```python
from build123d import *

# Parameters (mm, degrees)
BOSS_EXTRUDE1_DEPTH            = 5
SKETCH3_R                      = 4
BOSS_EXTRUDE2_DEPTH            = 5
CHAMFER1_SIZE                  = 1
M6X1_0_TAPPED_HOLE2_AT_2_COUNT = 2
M6X1_0_TAPPED_HOLE2_AT_2_PITCH = 0.000121298


with BuildPart() as part:
    # Sketch1 → Boss-Extrude1 (new, symmetric)
    with BuildSketch(Plane(origin=(0, 0, 0), x_dir=(1, 0, 0), z_dir=(0, 1, 0))):
        Polygon((0, 5.5), (-4.763139721, 2.75), (-4.763139721, -2.75), (0, -5.5), (4.763139721, -2.75), (4.763139721, 2.75), align=None)
    extrude(amount=BOSS_EXTRUDE1_DEPTH, both=True)

    # Sketch3 → Boss-Extrude2 (add)
    with BuildSketch(Plane(origin=(0, 5, 0), x_dir=(1, 0, 0), z_dir=(0, 1, 0))):
        with Locations(Location((0, 0, 0), (0, 0, 270))):
            Circle(SKETCH3_R)
    extrude(amount=BOSS_EXTRUDE2_DEPTH)

    # Chamfer1
    chamfer1_edges = [part.edges().sort_by_distance(p)[0] for p in [
        (0, 10, -4),
    ]]
    chamfer(chamfer1_edges, length=CHAMFER1_SIZE)

    # Sketch19 → M6x1.0 Tapped Hole2 (revolve, cut)
    with BuildSketch(Plane(origin=(-7.813e-06, -5, 0.000121047), x_dir=(0, 0, -1), z_dir=(1, 0, 0))):
        Polygon((0, 0), (0, 9.502151548), (2.5, 8), (2.5, 0), align=None)
    m6x1_0_tapped_hole2 = revolve(axis=Axis((-7.813e-06, -11.35, 0.000121047), (0, 1, 0)), mode=Mode.SUBTRACT)

    # M6x1.0 Tapped Hole2 at 2: M6x1.0 Tapped Hole2 ×2
    with Locations(*[Vector(0.06441225047789163, 0, -0.9979233748080929) * (i * M6X1_0_TAPPED_HOLE2_AT_2_PITCH) for i in range(1, M6X1_0_TAPPED_HOLE2_AT_2_COUNT)]):
        add(m6x1_0_tapped_hole2, mode=Mode.SUBTRACT)


solid = part.part
```
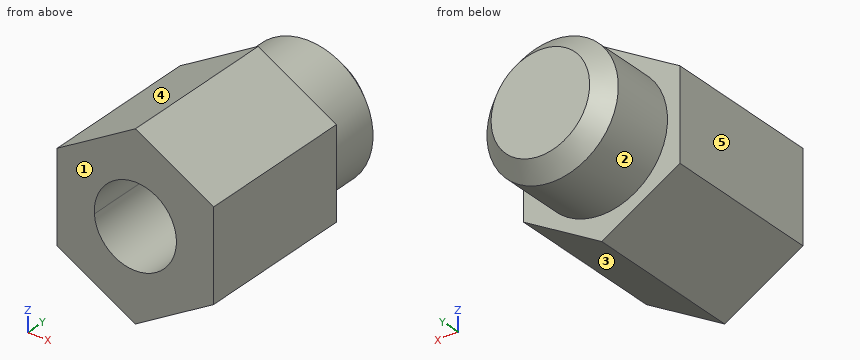
Geometry: final body of the model. Coordinates: model frame, mm. Face numbers are marked on the shaded views. A direction names the side the tool comes from. Coordinates: 2 decimals unless noted, no trailing zeros. Loops run counter-clockwise (first coordinate to the right, second up) from the corner with the lowest first, then second, coordinate; pieces in that order, holes last. Notation, with made-up numbers: (29.5, 5) -> (51.5, 5) arc R13 cw to (51.5, 17) -> close; hole circle Ø4 at (-34.5, -28.5). An arc over 180 degrees is marked (long way). Use a Markdown table: item, result. Add a question column.
(1) Access query for the marked faces 1 and 2. Directions: +Z, -Z, +X, -X, +Y, -Y. A direction counts if a zero-diameter tool reaches every point of the face in a straight line with its end or side. Return the directions, or none.
(2) Line query: line 1 along X through (y, z) = (0.25, 0); line 2 along X through (y, z) = (2, -1.5); line 3 along Z through (x, y) = (-0.75, -1.5). Output: solid intervals per line, ascending.
(3) Pin query (flat end, axial travel): pin 1 Ø2 at (x, z) = (-2.5, -2.5) entering from +Y; pin 2 Ø1.5 at (y, z) = (6.5, -2) entering from +X; pin 3 Ø1 at (y, z) = (3.5, -3.5) entering from -X. Return the tip coordinate at first contact, or that it passes through.
(4) Section query B-B, the plane z = 4.5. Return loops of the section in (x, y), plus the area to 3 significant figures.
(5) Mould query, pull axis Z, two halves, no side actions, for the marked faces 3, 4 and 5. Classes: pulls with the +Z half, pulls with the -Z half, needs draft (parallel to the pull), parting line crosses it, or undercut.
(6) Section query A-A, the plane y = 8.5. Return loops of the section in (x, z), plus the area to 3 significant figures.
Answer:
| question | item | result |
|---|---|---|
| 1 | face 1 | +Z, -Z, +X, -X, -Y |
| 1 | face 2 | +Y |
| 2 | line 1 | x = -4.76 to -2.5, 2.5 to 4.76 |
| 2 | line 2 | x = -4.76 to -2, 2 to 4.76 |
| 2 | line 3 | z = -5.07 to -2.38, 2.38 to 5.07 |
| 3 | pin 1 | stops at y = 10 |
| 3 | pin 2 | stops at x = 3.8 |
| 3 | pin 3 | stops at x = -4.33 |
| 4 | outline | (-1.73, -5) -> (1.73, -5) -> (1.73, 5) -> (-1.73, 5) -> close |
| 4 | area | 34.6 mm^2 |
| 5 | face 3 | pulls with the -Z half |
| 5 | face 4 | pulls with the +Z half |
| 5 | face 5 | needs draft |
| 6 | outline | circle Ø8 at (0, 0) |
| 6 | area | 50.3 mm^2 |
